Print and shaded views of the part. All mm, measured from the part's lowest x, y and z. A direction names the side the tool comes from. Give positions to 0.01 mm unless a question says otherwise; leave off trailing zeros. Write each loop counter-clockwise with the first axis right and the second up, starting at its lowest first coordinate (ties: lowest second). Pieces come first, ordered by that corner, then holes. Notation, with made-up numbers: (63, -13.5) -> (106, -13.5) arc R13 ccw to (106, -5.5) -> close; hole circle Ø1 at (77.5, -7.5). An arc over 180 degrees is marked (long way). Put each result on its own line as item: value.
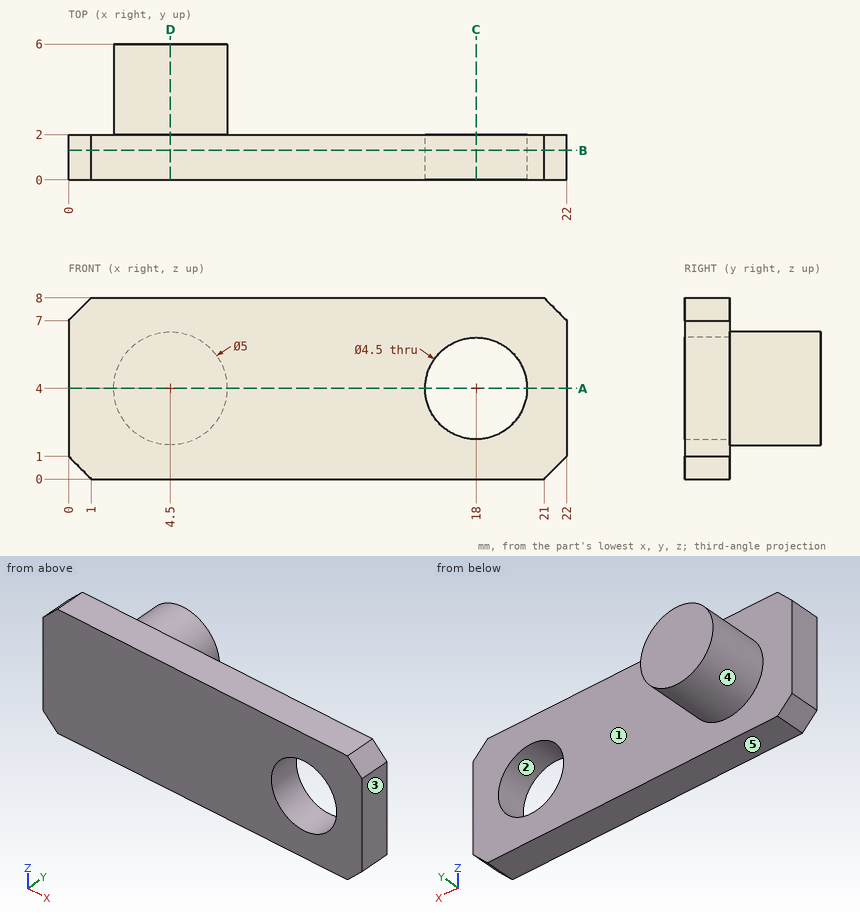
1) Pin check, flat tips, straight feed: pin 1 (1.5 mm diameter, centred on y = 3, z = 4, fed in from -X); pin 2 (4 mm diameter, centred on x = 18, z = 4, fed in from -Y). Stop position of each tip, or through.
Filled sheet:
pin 1: x = 2
pin 2: through
2) Wall check: L1, parallel to X at y = 0.7, z = 4; L2, parallel to Y at x = 12, z = 6.5; L3, parallel to X at y = 0.5, z = 3. Give the ranges that are in metal, low to high.
Filled sheet:
L1: 0 to 15.75, 20.25 to 22
L2: 0 to 2
L3: 0 to 15.98, 20.02 to 22
3) Slice it at C-C (x = 18). Write the cut outline in (y, z).
Filled sheet:
outline: (0, 0) -> (2, 0) -> (2, 1.75) -> (0, 1.75) -> close; (0, 6.25) -> (2, 6.25) -> (2, 8) -> (0, 8) -> close
4) Pull direction X, two halves, no side cores. Call the marked faces 1, 2 and 3: released by +X, released by -X, zero draft, split by the parting line, or undercut.
Filled sheet:
face 1: zero draft
face 2: undercut
face 3: released by +X
5) Slice it at A-A (z = 4). Write the cut outline in (x, y).
Filled sheet:
outline: (0, 0) -> (15.75, 0) -> (15.75, 2) -> (7, 2) -> (7, 6) -> (2, 6) -> (2, 2) -> (0, 2) -> close; (20.25, 0) -> (22, 0) -> (22, 2) -> (20.25, 2) -> close
6) Tool access for the marked faces 4 and 5: list every direction of +Z, -Z, +X, -X, +Y, -Y with a clear straight run to the whole face (end or side of a thin tool).
Filled sheet:
face 4: +Y
face 5: -Z, +X, -X, +Y, -Y
7) Slice it at B-B (y = 1.3). Write the cut outline in (x, z), plus the area to 3 significant figures.
Filled sheet:
outline: (0, 1) -> (1, 0) -> (21, 0) -> (22, 1) -> (22, 7) -> (21, 8) -> (1, 8) -> (0, 7) -> close; hole circle Ø4.5 at (18, 4)
area: 158 mm2
8) Slice it at D-D (x = 4.5). Write the cut outline in (y, z).
Filled sheet:
outline: (0, 0) -> (2, 0) -> (2, 1.5) -> (6, 1.5) -> (6, 6.5) -> (2, 6.5) -> (2, 8) -> (0, 8) -> close
